Geometry check sheet. Reference: drawing and pictorial views, mm from the part's lowest x, y, z. Coordinates: 2 decimals unless noted, no trailing zeros. Write each loop counter-clockwise with the first axis right and the second up, starting at its lowest first coordinate (ties: lowest second). Pieces come first, ordered by that corner, then holes. Notation, with made-up numbers: (-37, -19.75) - (-2, -19.75) arc R12 ccw to (-2, -13.75) - close; hole circle Ø4 at (-34.75, 87). An arc over 180 degrees is marked (long way). Answer as a JSON object with one key per item and string values. Group by question number.
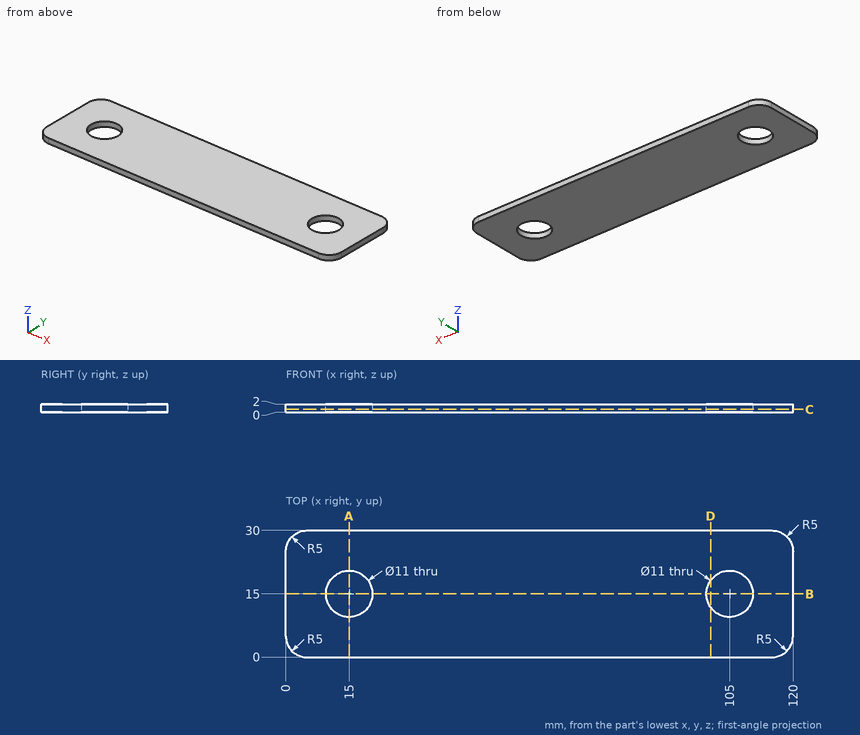
(1) Section check D-D (x = 100.5). Record the cut outline in (y, z), and give its area (3 significant figures).
(2) Section check B-B (y = 15). Record the cut outline in (x, z).
(3) Section check A-A (x = 15). Record the cut outline in (y, z).
(4) Material ranges on L1, parallel to X at y = 14.5, z = 0.7; L2, parallel to Y at x = 105, z = 0.5; L3, parallel to Y at x = 16, z = 0.65, recorded low to high. Write a range as [from, to].
(5) Section check C-C (z = 0.75). Record the cut outline in (x, y).
Conclusion:
{
 "1": {"outline": "(0, 0) - (11.84, 0) - (11.84, 2) - (0, 2) - close; (18.16, 0) - (30, 0) - (30, 2) - (18.16, 2) - close", "area": "47.4 mm^2"},
 "2": {"outline": "(0, 0) - (9.5, 0) - (9.5, 2) - (0, 2) - close; (20.5, 0) - (99.5, 0) - (99.5, 2) - (20.5, 2) - close; (110.5, 0) - (120, 0) - (120, 2) - (110.5, 2) - close"},
 "3": {"outline": "(0, 0) - (9.5, 0) - (9.5, 2) - (0, 2) - close; (20.5, 0) - (30, 0) - (30, 2) - (20.5, 2) - close"},
 "4": {"L1": "x = [0, 9.52], [20.48, 99.52], [110.48, 120]", "L2": "y = [0, 9.5], [20.5, 30]", "L3": "y = [0, 9.59], [20.41, 30]"},
 "5": {"outline": "(0, 5) arc R5 ccw to (5, 0) - (115, 0) arc R5 ccw to (120, 5) - (120, 25) arc R5 ccw to (115, 30) - (5, 30) arc R5 ccw to (0, 25) - close; hole circle Ø11 at (15, 15); hole circle Ø11 at (105, 15)"}
}
